Model file for the job. Use its own axes, mm. Coordinates: 2 decimals unless noted, no trailing zeros. Loops run counter-clockwise (first coordinate to the right, second up) from the corner with the lowest first, then second, coordinate; pieces in that order, holes last.
from build123d import *

# Parameters (mm, degrees)
BOSS_EXTRUDE1_DEPTH = 16


with BuildPart() as part:
    # Sketch1 → Boss-Extrude1 (new body)
    with BuildSketch(Plane.XY):
        with BuildLine():
            Line((0, 165), (194.920512906, 165))
            ThreePointArc((194.920512906, 165), (195.997551485, 164.963708463), (197.06970414, 164.854998488))
            Line((197.06970414, 164.854998488), (616.5, 108))
            Line((616.5, 108), (1056.5, 108))
            Line((1056.5, 108), (1056.5, -108))
            Line((1056.5, -108), (616.5, -108))
            Line((616.5, -108), (197.06970414, -164.854998488))
            ThreePointArc((197.06970414, -164.854998488), (195.997551485, -164.963708463), (194.920512906, -165))
            Line((194.920512906, -165), (0, -165))
            Line((0, -165), (0, 165))
        make_face()
    extrude(amount=BOSS_EXTRUDE1_DEPTH)


solid = part.part
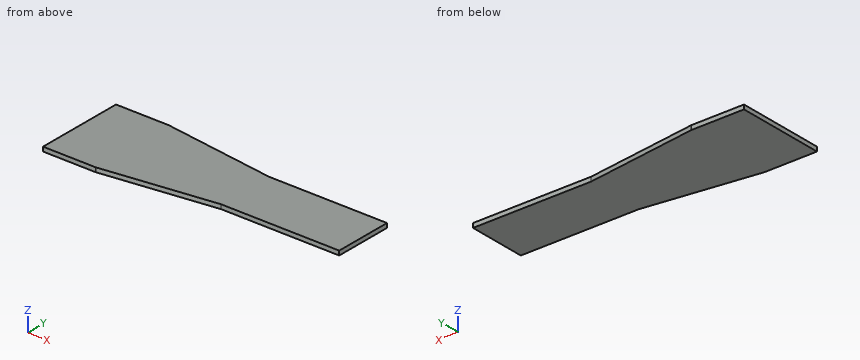
Q1. Slice it at C-C (y = 140.5). List the corners of the cut face in (x, z).
Answers:
outline: (0, 0) - (376.74, 0) - (376.74, 16) - (0, 16) - close
Q2. Slice it at A-A (z = 4.5). List the corners of the cut face in (x, y) (3 decimals), and give its area (3 significant figures).
Answers:
outline: (0, -165) - (194.921, -165) arc R16 ccw to (197.07, -164.855) - (616.5, -108) - (1056.5, -108) - (1056.5, 108) - (616.5, 108) - (197.07, 164.855) arc R16 ccw to (194.921, 165) - (0, 165) - close
area: 275,000 mm2
Q3. Flat gauge pin, fed straight in: P1, Ø8, axis at x = 851, z = 10, coming from the +Y side. Where does the tip first touch, or does it go through?
Answers:
P1: stops at y = 108
Q4. Slice it at B-B (x = 883). List the corners of the cut face in (y, z).
Answers:
outline: (-108, 0) - (108, 0) - (108, 16) - (-108, 16) - close
Q5. Drill centre lines: line 1 (Y direction, x = 771.5, z = 13.25); line 2 (Y direction, x = 195.5, z = 15.75). Where is each one in solid material? Low to high.
Answers:
line 1: y = -108 to 108
line 2: y = -164.99 to 164.99
